Geometry: final body of the model. Coordinates: model frame, mm. A direction names the side the tool comes from. Give positions to 0.01 mm unless a question says otherwise; leave off trailing zeros. Write each loop counter-clockwise with the first axis right and the second up, starting at its lowest first coordinate (ties: lowest second). Pieces come first, ordered by that corner, then holes. Notation, with made-up numbers: M 72.25,-6.5 L 91.25,-6.5 A11 cw 91.25,-2.5 Z; hole C 38,-18.5 d8. An arc over 180 degrees is marked long. Answer as a JSON object with one key per item and string values.
from build123d import *

# Parameters (mm, degrees)
SKETCH_1_W          = 370
SKETCH_1_H          = 440
EXTRUDE_1_DEPTH     = 5
CUT_EXTRUDE_1_REACH = 289.62
SKETCH_2_R          = 8
SKETCH_2_R_2        = 5.5
SKETCH_3_W          = 10
SKETCH_3_H          = 440
EXTRUDE_2_DEPTH     = 400
FILLET_1_R          = 40


with BuildPart() as part:
    # 草图1 → 凸台-拉伸1 (new, symmetric)
    with BuildSketch(Plane(origin=(0, 0, 0), x_dir=(1, 0, 0), z_dir=(0, 1, 0))):
        Rectangle(SKETCH_1_W, SKETCH_1_H)
    extrude(amount=EXTRUDE_1_DEPTH, both=True)

    # 草图2 → 切除-拉伸1 (cut, up to next)
    with BuildSketch(Plane(origin=(0, 5, 0), x_dir=(1, 0, 0), z_dir=(0, 1, 0)), mode=Mode.PRIVATE) as cut_extrude_1_sk1:
        with Locations(Location((0, 0, 0), (0, 0, 270))):
            Circle(SKETCH_2_R)
    cut_extrude_1_tool1 = extrude(cut_extrude_1_sk1.sketch, amount=-CUT_EXTRUDE_1_REACH, mode=Mode.PRIVATE) & part.part
    # 草图2 → 切除-拉伸1 (cut, up to next)
    with BuildSketch(Plane(origin=(0, 5, 0), x_dir=(1, 0, 0), z_dir=(0, 1, 0)), mode=Mode.PRIVATE) as cut_extrude_1_sk2:
        with Locations(Location((0, 150, 0), (0, 0, 270))):
            Circle(SKETCH_2_R_2)
    cut_extrude_1_tool2 = extrude(cut_extrude_1_sk2.sketch, amount=-CUT_EXTRUDE_1_REACH, mode=Mode.PRIVATE) & part.part
    # 草图2 → 切除-拉伸1 (cut, up to next)
    with BuildSketch(Plane(origin=(0, 5, 0), x_dir=(1, 0, 0), z_dir=(0, 1, 0)), mode=Mode.PRIVATE) as cut_extrude_1_sk3:
        with Locations(Location((0, -150, 0), (0, 0, 270))):
            Circle(SKETCH_2_R_2)
    cut_extrude_1_tool3 = extrude(cut_extrude_1_sk3.sketch, amount=-CUT_EXTRUDE_1_REACH, mode=Mode.PRIVATE) & part.part
    add(cut_extrude_1_tool1.solids().sort_by_distance((0, 5, 0))[0], mode=Mode.SUBTRACT)
    add(cut_extrude_1_tool2.solids().sort_by_distance((0, 5, -150))[0], mode=Mode.SUBTRACT)
    add(cut_extrude_1_tool3.solids().sort_by_distance((0, 5, 150))[0], mode=Mode.SUBTRACT)

    # 草图3 → 凸台-拉伸2 (add)
    with BuildSketch(Plane(origin=(0, 5, 0), x_dir=(1, 0, 0), z_dir=(0, 1, 0))):
        with Locations((-180, 0)):
            Rectangle(SKETCH_3_W, SKETCH_3_H)
    extrude(amount=EXTRUDE_2_DEPTH)

    # 圆角1
    fillet_1_edges = [part.edges().sort_by_distance(p)[0] for p in [
        (-180, 405, 220),
        (-180, 405, -220),
        (185, 0, 220),
        (185, 0, -220),
    ]]
    fillet(fillet_1_edges, radius=FILLET_1_R)


solid = part.part
1) Cut plane C-C on y = 56. Return loops of the section in (x, z), and give its area (3 significant figures).
Geometry check:
{"outline": "M -185,-220 L -175,-220 L -175,220 L -185,220 Z", "area": "4,400 mm2"}
2) Set-up query: faces 1 (the flat face through (42, 5, -3)), 2 (the flat face through (-44, -5, -3)). Return all of +Z, -Z, +X, -X, +Y, -Y with unobstructed straight access to the full face (end or side cutting, diameter ignored); none if empty.
Geometry check:
{"face 1": "+Z, -Z, +X, +Y", "face 2": "+Z, -Z, +X, -X, -Y"}
3) Cut plane A-A on z = 0. Return loops of the section in (x, y).
Geometry check:
{"outline": "M -185,-5 L -8,-5 L -8,5 L -175,5 L -175,405 L -185,405 Z; M 8,-5 L 185,-5 L 185,5 L 8,5 Z"}
4) Pull-direction query (X, two-part tool) for faces 3 (the cylindrical face through (172.972, 0.07, 208.594)), 4 (the flat face through (-180, 97, -220)), 5 (the cylindrical face through (0.242, 0.07, 144.505)); classes: pulls with the +X half, pulls with the -X half, needs draft (parallel to the pull), parting line crosses it, or undercut.
Geometry check:
{"face 3": "pulls with the +X half", "face 4": "needs draft", "face 5": "undercut"}
5) Cut plane D-D on x = 67. Return loops of the section in (y, z), and give its area (3 significant figures).
Geometry check:
{"outline": "M -5,-220 L 5,-220 L 5,220 L -5,220 Z", "area": "4,400 mm2"}
6) Contact query for flat-ended pins moving along their axis: P1, Ø14.5, axis at x = 0, z = -150, coming from the -Y side; P2, Ø3, axis at x = 56, z = 85, coming from the +Y side; P3, Ø10, axis at x = 0, z = 150, coming from the -Y side. Output: stop coordinate, or through.
Geometry check:
{"P1": "stops at y = -5", "P2": "stops at y = 5", "P3": "passes through"}
7) Cut plane B-B on z = -63. Return loops of the section in (x, y), and give its area (3 significant figures).
Geometry check:
{"outline": "M -185,-5 L 185,-5 L 185,5 L -175,5 L -175,405 L -185,405 Z", "area": "7,700 mm2"}
8) Line query: line 1 (X direction, y = 1, z = -150); line 2 (X direction, y = 1.5, z = 0); line 3 (Y direction, x = -92.5, z = 133.5). Output: solid intervals per line, ascending. Write a range as from..to.
Geometry check:
{"line 1": "x = -185..-5.5, 5.5..185", "line 2": "x = -185..-8, 8..185", "line 3": "y = -5..5"}
